from build123d import *

# Parameters (mm, degrees)
SKETCH1_R                                            = 19
BOSS_EXTRUDE1_DEPTH                                  = 45
SKETCH2_R                                            = 15
CUT_EXTRUDE1_DEPTH                                   = 30
M18X1_5_TAPPED_HOLE1_D                               = 16.5
M18X1_5_TAPPED_HOLE1_DEPTH                           = 43.5
M18X1_5_TAPPED_HOLE1_TIP                             = 4.957100107
BOSS_EXTRUDE2_START                                  = 10
SKETCH5_R                                            = 32
SKETCH5_R_2                                          = 15
BOSS_EXTRUDE2_DEPTH                                  = 10
HOLE_SIZE_PER_SOCKET_HEAD_CAP_SCREW_TYPE_D           = 4.5
HOLE_SIZE_PER_SOCKET_HEAD_CAP_SCREW_TYPE_CBORE_D     = 8
HOLE_SIZE_PER_SOCKET_HEAD_CAP_SCREW_TYPE_CBORE_DEPTH = 4.6
CIRPATTERN1_COUNT                                    = 6
CUT_EXTRUDE2_REACH                                   = 73.225
CHAMFER1_SIZE                                        = 1
CHAMFER2_SIZE                                        = 10
CHAMFER2_SIZE2                                       = 1.763269807
CHAMFER3_SIZE                                        = 1
CHAMFER3_SIZE2                                       = 1.232803052
CHAMFER4_SIZE                                        = 2


with BuildPart() as part:
    # Sketch1 → Boss-Extrude1 (new body)
    with BuildSketch(Plane.XY):
        with Locations(Location((0, 0, 0), (0, 0, 180))):
            Circle(SKETCH1_R)
    extrude(amount=BOSS_EXTRUDE1_DEPTH)

    # Sketch2 → Cut-Extrude1 (cut)
    with BuildSketch(Plane.XY.offset(45)):
        Circle(SKETCH2_R)
    extrude(amount=-CUT_EXTRUDE1_DEPTH, mode=Mode.SUBTRACT)

    # M18x1.5 Tapped Hole1
    with Locations(Plane(origin=(0, 0, 0), x_dir=(-1, 0, 0), z_dir=(0, 0, -1))):
        with Locations((0, 0)):
            Hole(M18X1_5_TAPPED_HOLE1_D / 2, depth=M18X1_5_TAPPED_HOLE1_DEPTH)
            with Locations((0, 0, -(M18X1_5_TAPPED_HOLE1_DEPTH + M18X1_5_TAPPED_HOLE1_TIP / 2))):  # 118° drill point
                Cone(0, M18X1_5_TAPPED_HOLE1_D / 2, M18X1_5_TAPPED_HOLE1_TIP, mode=Mode.SUBTRACT)

    # Sketch5 → Boss-Extrude2 (add)
    with BuildSketch(Plane.XY.offset(45).offset(BOSS_EXTRUDE2_START)):
        Circle(SKETCH5_R)
        Circle(SKETCH5_R_2, mode=Mode.SUBTRACT)
    extrude(amount=-BOSS_EXTRUDE2_DEPTH)

    # Hole size per socket head cap screw type1 (through all)
    with Locations(Plane(origin=(0, 25, 55), x_dir=(1, 0, 0), z_dir=(0, 0, 1))):
        with Locations((0, 0)):
            hole_size_per_socket_head_cap_screw_type = CounterBoreHole(HOLE_SIZE_PER_SOCKET_HEAD_CAP_SCREW_TYPE_D / 2, HOLE_SIZE_PER_SOCKET_HEAD_CAP_SCREW_TYPE_CBORE_D / 2, HOLE_SIZE_PER_SOCKET_HEAD_CAP_SCREW_TYPE_CBORE_DEPTH)

    # CirPattern1: Hole size per socket head cap screw type1 ×6 about axis, 2 skipped
    cirpattern1_axis = Axis((0, 0, 55), (0, 0, 1))
    add([hole_size_per_socket_head_cap_screw_type.rotate(cirpattern1_axis, i * 360 / CIRPATTERN1_COUNT) for i in range(1, CIRPATTERN1_COUNT) if i not in (1, 4)], mode=Mode.SUBTRACT)

    # Sketch7 → Cut-Extrude2 (cut, up to next)
    with BuildSketch(Plane.XY.offset(55), mode=Mode.PRIVATE) as cut_extrude2_sk1:
        with BuildLine():
            Line((-8.108511332, 30.955646399), (-30.862631838, -8.455646399))
            ThreePointArc((-30.862631838, -8.455646399), (-27.712812921, 16), (-8.108511332, 30.955646399))
        make_face()
    cut_extrude2_tool1 = extrude(cut_extrude2_sk1.sketch, amount=-CUT_EXTRUDE2_REACH, mode=Mode.PRIVATE) & part.part
    # Sketch7 → Cut-Extrude2 (cut, up to next)
    with BuildSketch(Plane.XY.offset(55), mode=Mode.PRIVATE) as cut_extrude2_sk2:
        with BuildLine():
            Line((30.862631838, 8.455646399), (8.108511332, -30.955646399))
            ThreePointArc((8.108511332, -30.955646399), (27.712812921, -16), (30.862631838, 8.455646399))
        make_face()
    cut_extrude2_tool2 = extrude(cut_extrude2_sk2.sketch, amount=-CUT_EXTRUDE2_REACH, mode=Mode.PRIVATE) & part.part
    add(cut_extrude2_tool1.solids().sort_by_distance((-22.822298, 13.17646, 55))[0], mode=Mode.SUBTRACT)
    add(cut_extrude2_tool2.solids().sort_by_distance((22.822298, -13.17646, 55))[0], mode=Mode.SUBTRACT)

    # Chamfer1
    chamfer1_edges = [part.edges().sort_by_distance(p)[0] for p in [
        (-16, -27.712812921, 55),
        (-16, -27.712812921, 45),
        (16, 27.712812921, 55),
        (16, 27.712812921, 45),
    ]]
    chamfer(chamfer1_edges, length=CHAMFER1_SIZE)

    # Chamfer2
    chamfer2_edges = [part.edges().sort_by_distance(p)[0] for p in [
        (19, 0, 0),
    ]]
    chamfer2_side = [part.faces().sort_by_distance(p)[0] for p in [
        (19, 0, 22.5),
    ]]
    chamfer(chamfer2_edges, length=CHAMFER2_SIZE, length2=CHAMFER2_SIZE2, reference=chamfer2_side[0])

    # Chamfer3
    chamfer3_edges = [part.edges().sort_by_distance(p)[0] for p in [
        (17.236730193, 0, 0),
    ]]
    chamfer3_side = [part.faces().sort_by_distance(p)[0] for p in [
        (18.118365096, 0, 5),
    ]]
    chamfer(chamfer3_edges, length=CHAMFER3_SIZE, length2=CHAMFER3_SIZE2, reference=chamfer3_side[0])

    # Chamfer4
    chamfer4_edges = [part.edges().sort_by_distance(p)[0] for p in [
        (-15, 0, 55),
    ]]
    chamfer(chamfer4_edges, length=CHAMFER4_SIZE)


solid = part.part
Could you check a few things on this model? Use its own coordinates, in mm. A direction names the side the tool comes from. Give positions to 0.01 mm unless a question says otherwise; leave off trailing zeros. Order: outer loops, then holes, each group sorted by start corner. A loop starts at its lowest first (then second) coordinate and runs counter-clockwise, first axis right, second up.
Item 1: If we mould it in two halves opening along X, with no side actions, what happens to faces 1 (the face through (-19.326, 11.526, 50.07)), 2 (the face through (2.3, -17.514, 2.424)), 3 (the face through (17.956, 14.032, 52.732)), 4 (the face through (-7, 7, 0))? For each: pulls with the +X half, pulls with the -X half, needs draft (parallel to the pull), parting line crosses it, or undercut.
Item 2: If we section it at A-A, the plane x = 0: Count the separate pieces of the cut face and the enclosed holes in it, plus the area to 3 significant figures.
Item 3: I need wall thicknesses on line 1 (Y direction, x = 0, z = 53); line 2 (X direction, y = 0.5, z = 44.5); line 3 (Y direction, x = 0, z = 53.2). Which ranges of each line are inside material? Lowest first, please.
Item 4: I'm going to push flat-ended pins straight in: pin 1 (5 mm diameter, centred on x = 0, y = 25, fed in from -Z); pin 2 (2 mm diameter, centred on x = -11.5, z = 41.5, fed in from +Y); pin 3 (9 mm diameter, centred on x = -4.5, y = 4.5, fed in from +Z). Where does each tip first touch, or does it pass through?
Item 5: For faces 5 (the face through (4.119, 18.548, 27.255)), 6 (the face through (-21, -10, 50.4)), 7 (the face through (7.62, -3.16, 7.61)), which set-ups out of +Z, -Z, +X, -X, +Y, -Y let a thin tool reach every point of the face, with its end or its side?
Item 6: If we section it at B-B, the plane z = 31: Write out the boundary of the cut face in (x, y).
Item 7: If we section it at C-C, the plane y = 0: Write out the boundary of the cut face in (x, z).
Values:
1. face 1: pulls with the -X half
1. face 2: parting line crosses it
1. face 3: undercut
1. face 4: needs draft
2. separate pieces: 4
2. enclosed holes: 0
2. area: 755 mm2
3. line 1: y = -32 to -29, -21 to -15, 15 to 21, 29 to 32
3. line 2: x = -18.99 to -14.99, 14.99 to 18.99
3. line 3: y = -32 to -29, -21 to -15.2, 15.2 to 21, 29 to 32
4. pin 1: stops at z = 45
4. pin 2: stops at y = 15.84
4. pin 3: stops at z = 15
5. face 5: -Z
5. face 6: +Z
5. face 7: +Z, -Z
6. outline: circle Ø38 at (0, 0); hole circle Ø30 at (0, 0)
7. outline: (-25.98, 45) - (-19, 45) - (-19, 10) - (-17.41, 0.98) - (-16, 0) - (-8.25, 0) - (-8.25, 15) - (-15, 15) - (-15, 53) - (-17, 55) - (-25.98, 55) - close; (8.25, 0) - (16, 0) - (17.41, 0.98) - (19, 10) - (19, 45) - (25.98, 45) - (25.98, 55) - (17, 55) - (15, 53) - (15, 15) - (8.25, 15) - close
